For this review, use the dimensioned drawing (mm, ordinates from the lowest corner) and the shaded views. A direction names the side the tool comes from. Give positions to 0.01 mm unless a question says otherwise; leave off trailing zeros. Loops run counter-clockwise (first coordinate to the right, second up) from the corner with the lowest first, then second, coordinate; pieces in that order, holes last. Notation, with made-up numbers: (38.25, 86.5) -> (59.25, 86.5) arc R31 cw to (59.25, 116.5) -> close; hole circle Ø11 at (25.25, 32). An arc over 180 degrees is marked (long way). Use a Markdown table: item, result. Add a question column.
1. Add section A-A (x = 3). State the section outline as (y, z) points, and give its area (3 significant figures).
2. For pin 1 Ø2.5 at (x, y) = (3.5, 4) entering from -Z; pin 2 Ø1 at (x, z) = (5, 32.5) entering from +Y; pin 3 Ø3 at (x, z) = (3, 21.5) entering from +Y, all flat-tipped, find the tip position at first contact; note any pin that passes through.
3. To check wall thickness, follow line 1 (Z direction, x = 2.55, y = 0.85); line 2 (X direction, y = 2.85, z = 18); line 3 (Z direction, x = 2.65, y = 5.7). State the ranges of each line that lie inside material, in increasing order.
4. Add section C-C (z = 9). State the section outline as (x, y) points.
5. For the marked faces 1 and 2, list the 3-axis set-ups (+Z, -Z, +X, -X, +Y, -Y) from which the entire face can be reached by the end or side of a thin tool; tool diameter is ignored.
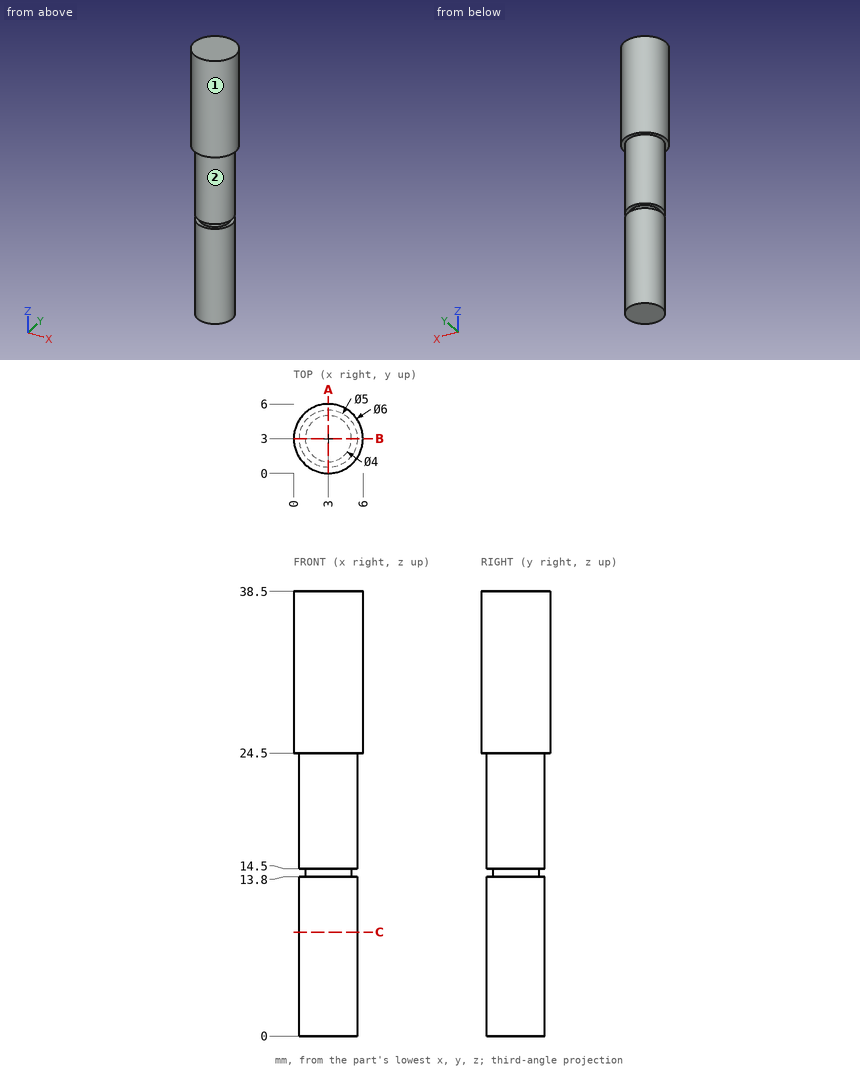
Taken from the geometry:
| question | item | result |
|---|---|---|
| 1 | outline | (0, 24.5) -> (0.5, 24.5) -> (0.5, 14.5) -> (1, 14.5) -> (1, 13.8) -> (0.5, 13.8) -> (0.5, 0) -> (5.5, 0) -> (5.5, 13.8) -> (5, 13.8) -> (5, 14.5) -> (5.5, 14.5) -> (5.5, 24.5) -> (6, 24.5) -> (6, 38.5) -> (0, 38.5) -> close |
| 1 | area | 206 mm^2 |
| 2 | pin 1 | stops at z = 0 |
| 2 | pin 2 | stops at y = 5.6 |
| 2 | pin 3 | stops at y = 5.5 |
| 3 | line 1 | z = 0 to 13.8, 14.5 to 38.5 |
| 3 | line 2 | x = 0.5 to 5.5 |
| 3 | line 3 | z = 24.5 to 38.5 |
| 4 | outline | circle Ø5 at (3, 3) |
| 5 | face 1 | +Z, -Z |
| 5 | face 2 | -Z |
